Input: part model. Units: mm. Frame: model coordinates. A direction names the side the tool comes from. Coordinates: 2 decimals unless noted, no trailing zeros. Loops run counter-clockwise (first coordinate to the right, second up) from the corner with the lowest first, then second, coordinate; pieces in that order, holes last.
```python
from build123d import *

# Parameters (mm, degrees)
SKETCH_1_W      = 64
SKETCH_1_H      = 38
EXTRUDE_1_DEPTH = 1
SKETCH_2_W      = 60
SKETCH_2_H      = 34
EXTRUDE_2_DEPTH = 9


with BuildPart() as part:
    # 草图1 → 凸台-拉伸1 (new, symmetric)
    with BuildSketch(Plane.XY):
        Rectangle(SKETCH_1_W, SKETCH_1_H)
    extrude(amount=EXTRUDE_1_DEPTH, both=True)

    # 草图2 → 凸台-拉伸2 (add)
    with BuildSketch(Plane.XY):
        Rectangle(SKETCH_2_W, SKETCH_2_H)
    extrude(amount=EXTRUDE_2_DEPTH)


solid = part.part
```
Item 1: Section query B-B (y = -14). Output: boundary loops of the cut face in (x, z).
Result:
outline: (-32, -1) - (32, -1) - (32, 1) - (30, 1) - (30, 9) - (-30, 9) - (-30, 1) - (-32, 1) - close
Item 2: Reachability of faces 1 (the face through (-30, 0, 5)), 2 (the face through (0, -17, 5)), 3 (the face through (30, 0, 5)) from +Z, -Z, +X, -X, +Y, -Y: full face, straight path, thin tool, end or side. Return the list, or none.
Result:
face 1: +Z, -X, +Y, -Y
face 2: +Z, +X, -X, -Y
face 3: +Z, +X, +Y, -Y
Item 3: Line query: L1, parallel to X at y = -10.5, z = 5.75; L2, parallel to Y at x = 7, z = 1.25. Output: solid intervals per line, ascending.
Result:
L1: x = -30 to 30
L2: y = -17 to 17
Item 4: Section query A-A (x = 15.5). Output: boundary loops of the cut face in (y, z), then the cut area to 3 significant figures.
Result:
outline: (-19, -1) - (19, -1) - (19, 1) - (17, 1) - (17, 9) - (-17, 9) - (-17, 1) - (-19, 1) - close
area: 348 mm2
Item 5: Contact query for a flat-ended pin moving along its axis: P1, Ø1.5, axis at x = -25, z = 2.5, coming from the +Y side. Output: stop coordinate, or through.
Result:
P1: stops at y = 17
Item 6: Section query C-C (z = 6). Output: boundary loops of the cut face in (x, y), then the cut area to 3 significant figures.
Result:
outline: (-30, -17) - (30, -17) - (30, 17) - (-30, 17) - close
area: 2,040 mm2
